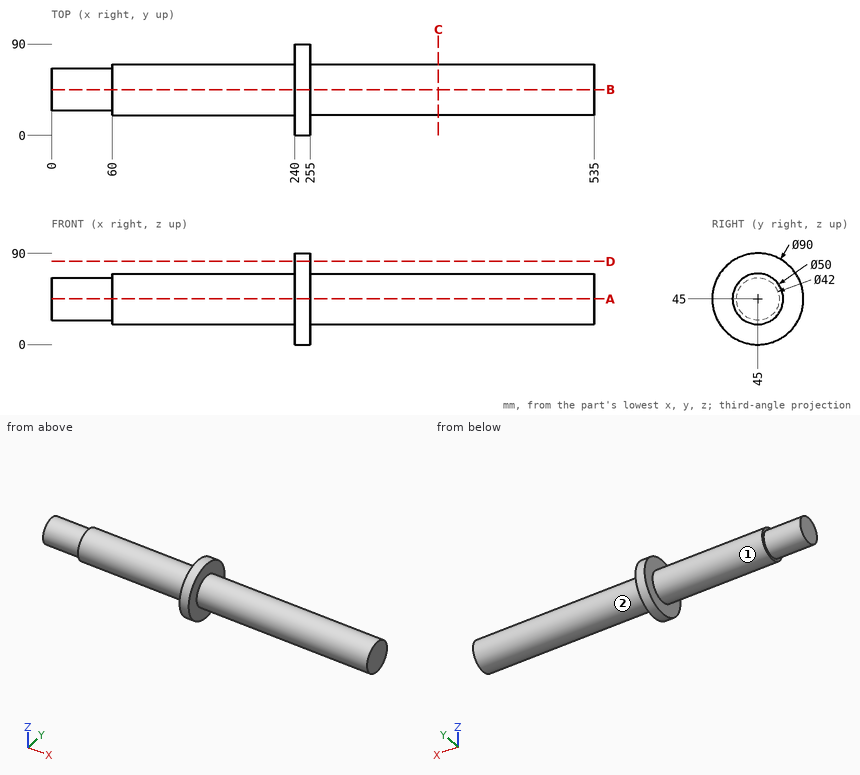
Could you check a few things on this drawing? It's one solid part, dimensions in mm from its lowest x, y, z. A direction names the side the tool comes from. Give positions to 0.01 mm unless a question says otherwise; leave off trailing zeros. Order: outer loops, then holes, each group sorted by start corner. A loop starts at its lowest first (then second) coordinate and runs counter-clockwise, first axis right, second up. Notation, with made-up numbers: (-24, 28) - (32, 28) arc R24 ccw to (32, 50) - close; hole circle Ø9 at (82.5, 30). An arc over 180 degrees is marked (long way). One line per question, with ' | ' between items. Start each with the question number.
Item 1: I want a section at C-C on x = 381.5. Write out the boundary of the cut face in (y, z).
Item 2: I want a section at D-D on z = 82. Write out the boundary of the cut face in (x, y).
Item 3: I'm going to push flat-ended pins straight in: pin 1 Ø6 at (x, z) = (126, 33.5) entering from +Y; pin 2 Ø3 at (y, z) = (73.5, 22.5) entering from +X; pin 3 Ø5 at (y, z) = (68.5, 73) entering from -X. Where does each tip first touch, or does it pass through?
Item 4: For the marked faces 1 and 2, which set-ups out of +Z, -Z, +X, -X, +Y, -Y let a thin tool reach every point of the face, with its end or its side?
Item 5: I need wall thicknesses on probe 1 along Z at (x, y) = (51, 45); probe 2 along X at (y, z) = (5, 38.5); probe 3 along Z at (x, y) = (70, 45.5) (3 decimals). Which ranges of each line are inside material? Lowest first, please. Write a range as [from, to].
Item 6: I want a section at A-A on z = 45. Write out the boundary of the cut face in (x, y), then the cut area to 3 significant figures.
Verdict:
1) outline: circle Ø50 at (45, 45)
2) outline: (240, 19.39) - (255, 19.39) - (255, 70.61) - (240, 70.61) - close
3) pin 1: y = 68.51 | pin 2: x = 255 | pin 3: x = 240
4) face 1: -X | face 2: +X
5) probe 1: [24, 66] | probe 2: [240, 255] | probe 3: [20.005, 69.995]
6) outline: (0, 24) - (60, 24) - (60, 20) - (240, 20) - (240, 0) - (255, 0) - (255, 20) - (535, 20) - (535, 70) - (255, 70) - (255, 90) - (240, 90) - (240, 70) - (60, 70) - (60, 66) - (0, 66) - close | area: 26,900 mm^2
